from build123d import *

# Parameters (mm, degrees)
SKETCH_1_W      = 22
SKETCH_1_H      = 36
SKETCH_1_R      = 1.45
EXTRUDE_1_DEPTH = 6.4
FILLET_1_R      = 1
FILLET_2_R      = 1


with BuildPart() as part:
    # 草图1 → 凸台-拉伸1 (new body)
    with BuildSketch(Plane(origin=(0, 0, 0), x_dir=(1, 0, 0), z_dir=(0, 1, 0))):
        Rectangle(SKETCH_1_W, SKETCH_1_H)
        with Locations(Location((-8, 15, 0), (0, 0, 270))):
            Circle(SKETCH_1_R, mode=Mode.SUBTRACT)
        with Locations(Location((8, 15, 0), (0, 0, 270))):
            Circle(SKETCH_1_R, mode=Mode.SUBTRACT)
        with Locations(Location((-8, -15, 0), (0, 0, 270))):
            Circle(SKETCH_1_R, mode=Mode.SUBTRACT)
        with Locations(Location((8, -15, 0), (0, 0, 270))):
            Circle(SKETCH_1_R, mode=Mode.SUBTRACT)
        with BuildLine():
            Line((-4.5, 15), (4.5, 15))
            ThreePointArc((4.5, 15), (5.525126266, 12.525126266), (8, 11.5))
            Line((8, 11.5), (8, -11.5))
            ThreePointArc((8, -11.5), (5.525126266, -12.525126266), (4.5, -15))
            Line((4.5, -15), (-4.5, -15))
            ThreePointArc((-4.5, -15), (-5.525126266, -12.525126266), (-8, -11.5))
            Line((-8, -11.5), (-8, 11.5))
            ThreePointArc((-8, 11.5), (-5.525126266, 12.525126266), (-4.5, 15))
        make_face(mode=Mode.SUBTRACT)
    extrude(amount=EXTRUDE_1_DEPTH)

    # 圆角1
    fillet_1_edges = [part.edges().sort_by_distance(p)[0] for p in [
        (8, 3.2, -11.5),
        (4.5, 3.2, -15),
        (-4.5, 3.2, -15),
        (-8, 3.2, -11.5),
        (-8, 3.2, 11.5),
        (-4.5, 3.2, 15),
        (4.5, 3.2, 15),
        (8, 3.2, 11.5),
    ]]
    fillet(fillet_1_edges, radius=FILLET_1_R)

    # 圆角2
    fillet_2_edges = [part.edges().sort_by_distance(p)[0] for p in [
        (-11, 3.2, -18),
        (11, 3.2, -18),
        (11, 3.2, 18),
        (-11, 3.2, 18),
    ]]
    fillet(fillet_2_edges, radius=FILLET_2_R)


solid = part.part
Could you check a few things on this model? Use its own coordinates, in mm. A direction names the side the tool comes from. Give positions to 0.01 mm unless a question says otherwise; leave off trailing zeros. Loops run counter-clockwise (first coordinate to the right, second up) from the corner with the lowest first, then second, coordinate; pieces in that order, holes last. Notation, with made-up numbers: (-3, 14.25) -> (3, 14.25) arc R10 ccw to (3, 33.25) -> close; hole circle Ø4 at (29.25, -21.75). An arc over 180 degrees is marked (long way). Answer as CSV lines item,"result". Start each with the question number.
(1) I need wall thicknesses on probe 1 along X at (y, z) = (1.5, -3.5); probe 2 along Z at (x, y) = (1, 2.5); probe 3 along X at (y, z) = (1.5, -11). Which ranges of each line are inside material? Lowest first, please.
(2) If we section it at B-B on y = 1.5: Write out the boundary of the cut face in (x, z).
(3) I'm going to push flat-ended pins straight in: pin 1 Ø3.5 at (x, z) = (-8, 15) entering from +Y; pin 2 Ø8 at (x, z) = (1, 5.5) entering from +Y. Where does each tip first touch, or does it pass through?
(4) If we section it at A-A on x = 0.5: Write out the boundary of the cut face in (y, z), then the cut area to 3 significant figures.
(5) We'd pull the mould along Z, two halves only. Please class faces 1 (the cylindrical face through (4.24, 3.24, -14.78)), 2 (the flat face through (10, 0, 0)), 3 (the cylindrical face through (-10.715, 3.245, -17.699)): released by +Z, released by -Z, zero draft, split by the parting line, or undercut.
(6) If we section it at C-C on z = -12.5: Write out the boundary of the cut face in (x, y).
(7) Which directions (+Z, -Z, +X, -X, +Y, -Y) give clear straight access to the entire face, cutting with the end or side of a thin tool? Please do faces 4 (the cylindrical face through (-10.715, 3.245, 17.699)), 5 (the cylindrical face through (-7.78, 3.24, -11.24)).
Computed:
1,probe 1,"x = -11 to -8, 8 to 11"
1,probe 2,"z = -18 to -15, 15 to 18"
1,probe 3,"x = -11 to -7.92, 7.92 to 11"
2,outline,"(-11, -17) arc R1 ccw to (-10, -18) -> (10, -18) arc R1 ccw to (11, -17) -> (11, 17) arc R1 ccw to (10, 18) -> (-10, 18) arc R1 ccw to (-11, 17) -> close; hole circle Ø2.9 at (-8, -15); hole circle Ø2.9 at (-8, 15); hole (-8, -10.61) arc R1 ccw to (-7.22, -11.59) arc R3.5 cw to (-4.59, -14.22) arc R1 ccw to (-3.61, -15) -> (3.61, -15) arc R1 ccw to (4.59, -14.22) arc R3.5 cw to (7.22, -11.59) arc R1 ccw to (8, -10.61) -> (8, 10.61) arc R1 ccw to (7.22, 11.59) arc R3.5 cw to (4.59, 14.22) arc R1 ccw to (3.61, 15) -> (-3.61, 15) arc R1 ccw to (-4.59, 14.22) arc R3.5 cw to (-7.22, 11.59) arc R1 ccw to (-8, 10.61) -> close; hole circle Ø2.9 at (8, -15); hole circle Ø2.9 at (8, 15)"
3,pin 1,"stops at y = 6.4"
3,pin 2,"passes through"
4,outline,"(0, -18) -> (6.4, -18) -> (6.4, -15) -> (0, -15) -> close; (0, 15) -> (6.4, 15) -> (6.4, 18) -> (0, 18) -> close"
4,area,"38.4 mm2"
5,face 1,"undercut"
5,face 2,"zero draft"
5,face 3,"released by -Z"
6,outline,"(-11, 0) -> (-5.55, 0) -> (-5.55, 6.4) -> (-11, 6.4) -> close; (5.55, 0) -> (11, 0) -> (11, 6.4) -> (5.55, 6.4) -> close"
7,face 4,"+Z, -X, +Y, -Y"
7,face 5,"+Y, -Y"
